For this review, take the finished solid that the model builds, in its own axes (mm). A direction names the side the tool comes from. Give positions to 0.01 mm unless a question says otherwise; leave off trailing zeros. Write each loop counter-clockwise with the first axis right and the second up, starting at its lowest first coordinate (ties: lowest second). Pieces come first, ordered by that corner, then holes. Notation, with made-up numbers: (86.5, -20.75) -> (111.5, -20.75) arc R22 cw to (111.5, -8.75) -> close; hole circle Ø6 at (-9, -19). An arc over 180 degrees is marked (long way). Answer as CSV lines item,"result".
```python
from build123d import *

# Parameters (mm, degrees)
CUT_EXTRUDE1_DEPTH = 2
CHAMFER1_SIZE      = 0.5


with BuildPart() as part:
    # Sketch1 → Revolve1 (revolve)
    with BuildSketch(Plane.XY, mode=Mode.PRIVATE) as revolve1_sk:
        Polygon((0, 0), (0, 19.5), (-4.5, 19.5), (-4.5, 16), (-2.5, 16), (-2.5, 8), (-2, 8), (-2, 0), align=None)
    revolve(revolve1_sk.sketch.rotate(Axis((0, 0, 0), (0, 1, 0)), 180), axis=Axis((0, 0, 0), (0, 1, 0)))

    # Sketch2 → Cut-Extrude1 (cut)
    with BuildSketch(Plane(origin=(0, 19.5, 0), x_dir=(1, 0, 0), z_dir=(0, 1, 0))):
        Polygon((1.50956506, 0.849242799), (0.019316692, 1.73194309), (-1.490248367, 0.882700291), (-1.50956506, -0.849242799), (-0.019316692, -1.73194309), (1.490248367, -0.882700291), align=None)
    extrude(amount=-CUT_EXTRUDE1_DEPTH, mode=Mode.SUBTRACT)

    # Chamfer1
    chamfer1_edges = [part.edges().sort_by_distance(p)[0] for p in [
        (-4.5, 16, 0),
        (-4.5, 19.5, 0),
    ]]
    chamfer(chamfer1_edges, length=CHAMFER1_SIZE)


solid = part.part
```
Q1. Add section A-A (z = 0). Write out the cut boundary in (x, y).
Answer block:
outline,"(-4.5, 16.5) -> (-4, 16) -> (-2.5, 16) -> (-2.5, 8) -> (-2, 8) -> (-2, 0) -> (2, 0) -> (2, 8) -> (2.5, 8) -> (2.5, 16) -> (4, 16) -> (4.5, 16.5) -> (4.5, 19) -> (4, 19.5) -> (1.5, 19.5) -> (1.5, 17.5) -> (-1.5, 17.5) -> (-1.5, 19.5) -> (-4, 19.5) -> (-4.5, 19) -> close"
Q2. Clearance check with flat-ended pins moving along their axes: pin 1 (1 mm diameter, centred on x = 1, y = 3, fed in from +Z); pin 2 (1 mm diameter, centred on y = 13.5, z = -2.5, fed in from -X); pin 3 (1 mm diameter, centred on y = 17, z = -1.5, fed in from +X). State where each tip first meets the part, or that it passes through.
Answer block:
pin 1,"stops at z = 1.94"
pin 2,"stops at x = -1.5"
pin 3,"stops at x = 4.39"
Q3. For faces 4 (the flat face through (0, 17.5, 0)), 5 (the flat face through (-1, 8, -2)), 6 (the cylindrical face through (-3.32, 17.73, -3.04)), list the 3-axis set-ups (+Z, -Z, +X, -X, +Y, -Y) from which the entire face can be reached by the end or side of a thin tool; tool diameter is ignored.
Answer block:
face 4,"+Y"
face 5,"-Y"
face 6,"+Y, -Y"
Q4. Add section B-B (y = 12). Write out the cut boundary in (x, z), plus the area to 3 significant figures.
Answer block:
outline,"circle Ø5 at (0, 0)"
area,"19.6 mm2"
Q5. Draft analysis for pull direction Z (two halves, no side actions). For faces 1 (the cylindrical face through (-2.5, 11.9, -0.1)), 2 (the flat face through (0, 0, 0)), 3 (the flat face through (0.725, 18.514, 1.313)), state which applies: released by +Z, released by -Z, zero draft, split by the parting line, or undercut.
Answer block:
face 1,"split by the parting line"
face 2,"zero draft"
face 3,"undercut"
Q6. To check wall thickness, follow probe 1 along Y at (x, z) = (-0.25, 1.25); probe 2 along Z at (x, y) = (0, 5.5); probe 3 along Y at (x, z) = (-1.5, 3.25). State the ranges of each line that lie inside material, in increasing order. Write a range as [from, to].
Answer block:
probe 1,"y = [0, 17.5]"
probe 2,"z = [-2, 2]"
probe 3,"y = [16, 19.5]"
